```python
from build123d import *

# Parameters (mm, degrees)
SKETCH_1_W                  = 150
SKETCH_1_H                  = 133
EXTRUDE_1_DEPTH             = 15
SKETCH_2_W                  = 32.584056601
SKETCH_2_H                  = 28.363937547
CUT_EXTRUDE_1_DEPTH         = 165.764225486
FILLET_8_R                  = 5
HOLE_WIZARD_1_D             = 5.3
HOLE_WIZARD_1_CBORE_D       = 10
HOLE_WIZARD_1_CBORE_DEPTH   = 5.7
HOLE_WIZARD_M4_3_D          = 3.3
HOLE_WIZARD_M4_3_DEPTH      = 15.5
HOLE_WIZARD_M4_3_TIP        = 0.991420021
SKETCH_20_W                 = 431.741055117
SKETCH_20_H                 = 139.105675049
CUT_EXTRUDE_5_DEPTH         = 15
SKETCH_24_W                 = 30
SKETCH_24_H                 = 177.502907688
CUT_EXTRUDE_6_DEPTH         = 5
HOLE_WIZARD_M4_2_D          = 3.3
HOLE_WIZARD_M4_2_DEPTH      = 11.5
HOLE_WIZARD_M4_2_TIP        = 0.991420021
HOLE_WIZARD_M4_1_AT_2_COUNT = 2
HOLE_WIZARD_M4_1_AT_2_PITCH = 40


with BuildPart() as part:
    # 草图1 → 凸台-拉伸1 (new body)
    with BuildSketch(Plane.XY):
        Rectangle(SKETCH_1_W, SKETCH_1_H)
    extrude(amount=EXTRUDE_1_DEPTH)

    # 草图2 → 切除-拉伸1 (cut, through all)
    with BuildSketch(Plane(origin=(75, 0, 0), x_dir=(0, 0, -1), z_dir=(1, 0, 0))):
        with Locations((-22.292028301, 78.681968774)):
            Rectangle(SKETCH_2_W, SKETCH_2_H)
    extrude(amount=-CUT_EXTRUDE_1_DEPTH, mode=Mode.SUBTRACT)

    # 圆角8
    fillet_8_edges = [part.edges().sort_by_distance(p)[0] for p in [
        (75, 66.5, 3),
        (-75, 66.5, 3),
        (-75, -66.5, 7.5),
        (75, -66.5, 7.5),
        (0, -66.5, 0),
        (-75, 0, 0),
        (75, 0, 0),
        (0, 66.5, 0),
    ]]
    fillet(fillet_8_edges, radius=FILLET_8_R)

    # 打孔尺寸(%根据)开槽圆柱头螺钉的类型1 (through all)
    with Locations(Plane(origin=(0, 0, 0), x_dir=(-1, 0, 0), z_dir=(0, 0, -1))):
        with Locations((0, 49.5), (0, -38.5)):
            CounterBoreHole(HOLE_WIZARD_1_D / 2, HOLE_WIZARD_1_CBORE_D / 2, HOLE_WIZARD_1_CBORE_DEPTH)

    # M4 螺纹孔3
    with Locations(Plane(origin=(0, 64.5, 0), x_dir=(1, 0, 0), z_dir=(0, 1, 0))):
        with Locations((0, -10.5), (66.5, -10.5), (-66.5, -10.5)):
            Hole(HOLE_WIZARD_M4_3_D / 2, depth=HOLE_WIZARD_M4_3_DEPTH)
            with Locations((0, 0, -(HOLE_WIZARD_M4_3_DEPTH + HOLE_WIZARD_M4_3_TIP / 2))):  # 118° drill point
                Cone(0, HOLE_WIZARD_M4_3_D / 2, HOLE_WIZARD_M4_3_TIP, mode=Mode.SUBTRACT)

    # 草图20 → 切除-拉伸5 (cut)
    with BuildSketch(Plane.XZ.offset(66.5)):
        with Locations((-98.598792732, 75.552837525)):
            Rectangle(SKETCH_20_W, SKETCH_20_H)
    extrude(amount=-CUT_EXTRUDE_5_DEPTH, mode=Mode.SUBTRACT)

    # 草图24 → 切除-拉伸6 (cut)
    with BuildSketch(Plane.XY.offset(15)):
        with Locations((-45, -6.351602415)):
            Rectangle(SKETCH_24_W, SKETCH_24_H)
    extrude(amount=-CUT_EXTRUDE_6_DEPTH, mode=Mode.SUBTRACT)

    # M4 螺纹孔2
    with Locations(Plane(origin=(0, -51.5, 0), x_dir=(-1, 0, 0), z_dir=(0, -1, 0))):
        with Locations((66.5, -10.5), (0, -10.5), (-66.5, -10.5)):
            Hole(HOLE_WIZARD_M4_2_D / 2, depth=HOLE_WIZARD_M4_2_DEPTH)
            with Locations((0, 0, -(HOLE_WIZARD_M4_2_DEPTH + HOLE_WIZARD_M4_2_TIP / 2))):  # 118° drill point
                Cone(0, HOLE_WIZARD_M4_2_D / 2, HOLE_WIZARD_M4_2_TIP, mode=Mode.SUBTRACT)

    # 草图28 → M4 螺纹孔1 (revolve, cut)
    with BuildSketch(Plane(origin=(75, 26.61076125, 10), x_dir=(0, 0, -1), z_dir=(0, 1, 0))):
        Polygon((0, 0), (0, 12.991420021), (1.65, 12), (1.65, 0), align=None)
    hole_wizard_m4_1 = revolve(axis=Axis((81.35, 26.61076125, 10), (-1, 0, 0)), mode=Mode.SUBTRACT)

    # M4 螺纹孔1 at 2: M4 螺纹孔1 ×2
    with Locations(*[(0, -i * HOLE_WIZARD_M4_1_AT_2_PITCH, 0) for i in range(1, HOLE_WIZARD_M4_1_AT_2_COUNT)]):
        add(hole_wizard_m4_1, mode=Mode.SUBTRACT)

    # 镜向1: M4 螺纹孔1 across plane
    add(hole_wizard_m4_1.mirror(Plane(origin=(0, 0, 0), x_dir=(0, 0, 1), z_dir=(1, 0, 0))), mode=Mode.SUBTRACT)

    # 镜向1 copy 1 sketch → 镜向1 copy 1 (revolve, cut)
    with BuildSketch(Plane(origin=(-75, -13.38923875, 10), x_dir=(0, 0, -1), z_dir=(0, 1, 0))):
        Polygon((0, 0), (0, -12.991420021), (1.65, -12), (1.65, 0), align=None)
    revolve(axis=Axis((-81.35, -13.38923875, 10), (-1, 0, 0)), mode=Mode.SUBTRACT)


solid = part.part
```
Source: CAD feature listing. Evaluate the final solid. Frame: model axes, mm. A direction names the side the tool comes from. Coordinates: 2 decimals unless noted, no trailing zeros. Loops run counter-clockwise (first coordinate to the right, second up) from the corner with the lowest first, then second, coordinate; pieces in that order, holes last. Notation, with made-up numbers: M 38.5,11 L 76.5,11 A24 ccw 76.5,43 Z; hole C -11,-16.5 d9. An arc over 180 degrees is marked long. Put each result on its own line as item: value. Start each with the question number.
1) Ray query, L1, parallel to X at y = 54.25, z = 10.5; L2, parallel to Y at x = 72, z = 10; L3, parallel to X at y = 37.5, z = 11.75. Return the intervals inside material, ascending. Write a range as from..to.
2) Contact query for flat-ended pins moving along their axis: pin 1 Ø1.5 at (x, z) = (-25, 9.5) entering from -Y; pin 2 Ø2.5 at (x, z) = (0, 10.5) entering from +Y; pin 3 Ø4.5 at (x, y) = (-33.5, -60) entering from +Z. Output: stop coordinate, or through.
3) Cut plane C-C on z = 1.75. Return the cut outline in (x, y).
4) Cut plane A-A on x = -42. Return the cut outline in (y, z).
5) Cut plane B-B on y = 4.5. Return the cut outline in (x, z).
6) Reachability of faces 4 (the face through (0.4, 57.9, 12.1)), 5 (the face through (1.524, -45.96, 11.132)), 6 (the face through (-69.084, -12.757, 8.476)), 7 (the face through (69.084, 24.975, 10.215)), 8 (the face through (0.651, 54.457, 2.81)) from +Z, -Z, +X, -X, +Y, -Y: full face, straight path, thin tool, end or side. Return the list, or none.
7) Pull-direction query (Y, two-part tool) for faces 1 (the face through (-62.181, 26.865, 9.868)), 2 (the face through (-1, -59, 6)), 3 (the face through (0.98, 65, 1.43)); classes: pulls with the +Y half, pulls with the -Y half, needs draft (parallel to the pull), parting line crosses it, or undercut.
The answers:
1. L1: x = -75..-68.15, -64.85..-60, -30..-1.65, 1.65..64.85, 68.15..75
1. L2: y = -51.5..-15.04, -11.74..24.96, 28.26..64.5
1. L3: x = -75..-60, -30..75
2. pin 1: stops at y = -51.5
2. pin 2: stops at y = 47.16
2. pin 3: stops at z = 6
3. outline: M -73.8,-61.5 A3.8 ccw -70,-65.3 L 70,-65.3 A3.8 ccw 73.8,-61.5 L 73.8,61.5 A3.8 ccw 70,65.3 L -70,65.3 A3.8 ccw -73.8,61.5 Z; hole C 0,-38.5 d10; hole C 0,49.5 d10
4. outline: M -66.5,5 A5 ccw -61.5,0 L 61.5,0 A5 ccw 66.5,5 L 66.5,6 L 64.5,6 L 64.5,10 L -51.5,10 L -51.5,6 L -66.5,6 Z
5. outline: M -75,5 A5 ccw -70,0 L 70,0 A5 ccw 75,5 L 75,15 L -30,15 L -30,10 L -60,10 L -60,15 L -75,15 Z
6. face 4: +Y
6. face 5: -Y
6. face 6: -X
6. face 7: +X
6. face 8: -Z
7. face 1: undercut
7. face 2: needs draft
7. face 3: pulls with the +Y half
